Build history of the part. All positions in model axes, mm. Round coordinates to 2 decimals unless told otherwise and drop trailing zeros. Write each loop counter-clockwise with the first axis right and the second up, starting at its lowest first coordinate (ties: lowest second). Pieces come first, ordered by that corner, then holes. Notation, with made-up numbers: (20.25, 89.5) -> (41.25, 89.5) arc R33 ccw to (41.25, 120.5) -> close; hole circle Ø10 at (-37.75, 72). An arc over 180 degrees is marked (long way). Answer in a Markdown table with one row per item.
```python
from build123d import *

# Parameters (mm, degrees)
BOSS_EXTRUDE1_DEPTH     = 5
SKETCH2_OUTSIDE_W       = 43.226
SKETCH2_OUTSIDE_H       = 46.71
SKETCH2_OUTSIDE_R       = 11.258330249
CUT_EXTRUDE1_DEPTH      = 10
CUT_EXTRUDE1_DRAFT      = -30
MIRROR1_COPY_1_SKETCH_W = 43.226
MIRROR1_COPY_1_SKETCH_H = 46.71
MIRROR1_COPY_1_SKETCH_R = 11.258330249
MIRROR1_COPY_1_DEPTH    = 10
MIRROR1_COPY_1_DRAFT    = -30
M12_TAPPED_HOLE3_D      = 10.2
M12_TAPPED_HOLE3_DEPTH  = 38.75


with BuildPart() as part:
    # Sketch1 → Boss-Extrude1 (new, symmetric)
    with BuildSketch(Plane.XY):
        Polygon((0, 13), (-11.258330249, 6.5), (-11.258330249, -6.5), (0, -13), (11.258330249, -6.5), (11.258330249, 6.5), align=None)
    extrude(amount=BOSS_EXTRUDE1_DEPTH, both=True)


with BuildPart() as cut_extrude1_tool:
    # Sketch2 outside → Cut-Extrude1 (with draft: the straight prism first)
    with BuildSketch(Plane.XY.offset(5)):
        Rectangle(SKETCH2_OUTSIDE_W, SKETCH2_OUTSIDE_H)
        Circle(SKETCH2_OUTSIDE_R, mode=Mode.SUBTRACT)
    extrude(amount=-CUT_EXTRUDE1_DEPTH)
    # Cut-Extrude1: the draft: its side faces are tilted about the plane it starts from
    cut_extrude1_sides = [cut_extrude1_tool.faces().sort_by_distance(p)[0] for p in [
        (0, -23.355, 0),
        (21.613, 0, 0),
        (0, 23.355, 0),
        (-21.613, 0, 0),
        (-11.258330249, 0, 0),
    ]]
    draft(cut_extrude1_sides, Plane.XY.offset(5), CUT_EXTRUDE1_DRAFT)


with BuildPart() as part_1:
    add(part.part)

    # Cut-Extrude1: cut by cut_extrude1_tool
    add(cut_extrude1_tool.part, mode=Mode.SUBTRACT)


with BuildPart() as mirror1_copy_1_tool:
    # Mirror1 copy 1 sketch → Mirror1 copy 1 (with draft: the straight prism first)
    with BuildSketch(Plane(origin=(0, 0, -5), x_dir=(1, 0, 0), z_dir=(0, 0, -1))):
        Rectangle(MIRROR1_COPY_1_SKETCH_W, MIRROR1_COPY_1_SKETCH_H)
        Circle(MIRROR1_COPY_1_SKETCH_R, mode=Mode.SUBTRACT)
    extrude(amount=-MIRROR1_COPY_1_DEPTH)
    # Mirror1 copy 1: the draft: its side faces are tilted about the plane it starts from
    mirror1_copy_1_sides = [mirror1_copy_1_tool.faces().sort_by_distance(p)[0] for p in [
        (0, -23.355, 0),
        (21.613, 0, 0),
        (0, 23.355, 0),
        (-21.613, 0, 0),
        (-11.258330249, 0, 0),
    ]]
    draft(mirror1_copy_1_sides, Plane(origin=(0, 0, -5), x_dir=(1, 0, 0), z_dir=(0, 0, -1)), MIRROR1_COPY_1_DRAFT)


with BuildPart() as part_2:
    add(part_1.part)

    # Mirror1 copy 1: cut by mirror1_copy_1_tool
    add(mirror1_copy_1_tool.part, mode=Mode.SUBTRACT)

    # M12 Tapped Hole3
    with Locations(Plane.XY.offset(5)):
        with Locations((0, 0)):
            Hole(M12_TAPPED_HOLE3_D / 2, depth=M12_TAPPED_HOLE3_DEPTH)


solid = part_2.part
```
Q1. Saw through at B-B on z = 2.75. Write the cut outline in (x, y).
A:
| item | result |
|---|---|
| outline | (-11.26, -5.56) arc R12.56 ccw to (-10.45, -6.97) -> (-0.81, -12.53) arc R12.56 ccw to (0.81, -12.53) -> (10.45, -6.97) arc R12.56 ccw to (11.26, -5.56) -> (11.26, 5.56) arc R12.56 ccw to (10.45, 6.97) -> (0.81, 12.53) arc R12.56 ccw to (-0.81, 12.53) -> (-10.45, 6.97) arc R12.56 ccw to (-11.26, 5.56) -> close; hole circle Ø10.2 at (0, 0) |
Q2. Drop flat-ended pins along their axis: P1, Ø4, axis at y = -9, z = 0.5, coming from the +X side; P2, Ø3, axis at x = -7.5, z = 0, coming from the -Y side; P3, Ø8, axis at x = 0, y = 0, coming from the -Z side. Give the stop position or say it passes through.
A:
| item | result |
|---|---|
| P1 | x = 10.39 |
| P2 | y = -9.54 |
| P3 | through |
Q3. Saw through at A-A on z = 1.25. Write the cut outline in (x, y).
A:
| item | result |
|---|---|
| outline | (-11.26, -6.5) -> (0, -13) -> (11.26, -6.5) -> (11.26, 6.5) -> (0, 13) -> (-11.26, 6.5) -> close; hole circle Ø10.2 at (0, 0) |
Q4. Two-plate mould, pull along Y, no slides. Class faces 1 (the flat face through (-5.55, 9.795, 0.07)), 2 (the flat face through (-11.258, 0, 0)), 3 (the cylindrical face through (-2.4, -4.5, -0.1)): released by +Y, released by -Y, zero draft, split by the parting line, or undercut.
A:
| item | result |
|---|---|
| face 1 | released by +Y |
| face 2 | zero draft |
| face 3 | undercut |
Q5. Wall check: line 1 (Y direction, x = 0, z = 2); line 2 (Y direction, x = 4, z = 4.75); line 3 (X direction, y = 4, z = 2). Give the ranges that are in metal, low to high. Write a range as [from, to].
A:
| item | result |
|---|---|
| line 1 | [-12.99, -5.1], [5.1, 12.99] |
| line 2 | [-10.68, -3.16], [3.16, 10.68] |
| line 3 | [-11.26, -3.16], [3.16, 11.26] |
Q6. Saw through at C-C on z = -4. Write the cut outline in (x, y), plus the area to 3 significant figures.
A:
| item | result |
|---|---|
| outline | (-11.26, -3.65) arc R11.84 ccw to (-8.79, -7.92) -> (-2.47, -11.58) arc R11.84 ccw to (2.47, -11.58) -> (8.79, -7.92) arc R11.84 ccw to (11.26, -3.65) -> (11.26, 3.65) arc R11.84 ccw to (8.79, 7.92) -> (2.47, 11.58) arc R11.84 ccw to (-2.47, 11.58) -> (-8.79, 7.92) arc R11.84 ccw to (-11.26, 3.65) -> close; hole circle Ø10.2 at (0, 0) |
| area | 341 mm² |
